from build123d import *

# Parameters (mm, degrees)
SKETCH1_W              = 200
SKETCH1_H              = 60
BOSS_EXTRUDE1_DEPTH    = 12
SKETCH2_W              = 16
SKETCH2_H              = 12
CUT_EXTRUDE1_DEPTH     = 106.090437243
SKETCH3_W              = 58
SKETCH3_H              = 28
CUT_EXTRUDE2_DEPTH     = 106.090437243
SKETCH4_W              = 58
SKETCH4_H              = 28
CUT_EXTRUDE3_DEPTH     = 106.090437243
SKETCH5_W              = 90
SKETCH5_H              = 5
M6_TAPPED_HOLE1_D      = 5
M6_TAPPED_HOLE1_DEPTH  = 13
M6_TAPPED_HOLE1_TIP    = 1.502151548
CHAMFER1_SIZE          = 1
CHAMFER2_SIZE          = 10
CHAMFER3_SIZE          = 5
FILLET1_R              = 10
M10_TAPPED_HOLE1_D     = 8.5
M10_TAPPED_HOLE1_DEPTH = 99.5
M10_TAPPED_HOLE1_TIP   = 2.553657631


with BuildPart() as part:
    # Sketch1 → Boss-Extrude1 (new body)
    with BuildSketch(Plane.XY.offset(6)):
        Rectangle(SKETCH1_W, SKETCH1_H)
    extrude(amount=-BOSS_EXTRUDE1_DEPTH)

    # Sketch2 → Cut-Extrude1 (cut, through all)
    with BuildSketch(Plane(origin=(0, 0, -6), x_dir=(-1, 0, 0), z_dir=(0, 0, -1))):
        with Locations((92, 0)):
            Rectangle(SKETCH2_W, SKETCH2_H)
    extrude(amount=-CUT_EXTRUDE1_DEPTH, mode=Mode.SUBTRACT)

    # Sketch3 → Cut-Extrude2 (cut, through all)
    with BuildSketch(Plane.XY.offset(6)):
        with Locations((-22, 0.2)):
            Rectangle(SKETCH3_W, SKETCH3_H)
    extrude(amount=-CUT_EXTRUDE2_DEPTH, mode=Mode.SUBTRACT)

    # Sketch4 → Cut-Extrude3 (cut, through all)
    with BuildSketch(Plane(origin=(0, 0, -6), x_dir=(-1, 0, 0), z_dir=(0, 0, -1))):
        with Locations((-58, 0.2)):
            Rectangle(SKETCH4_W, SKETCH4_H)
    extrude(amount=-CUT_EXTRUDE3_DEPTH, mode=Mode.SUBTRACT)

    # Sketch5 → Revolve1 (revolve)
    with BuildSketch(Plane(origin=(0, 0, 0), x_dir=(-1, 0, 0), z_dir=(0, 0, -1)), mode=Mode.PRIVATE) as revolve1_sk:
        with Locations((-145, 2.7)):
            Rectangle(SKETCH5_W, SKETCH5_H)
    revolve(revolve1_sk.sketch.rotate(Axis((190, 0.2, 0), (-1, 0, 0)), 270), axis=Axis((190, 0.2, 0), (-1, 0, 0)))

    # M6 Tapped Hole1
    with Locations(Plane.ZY.offset(100)):
        with Locations((0, 18)):
            Hole(M6_TAPPED_HOLE1_D / 2, depth=M6_TAPPED_HOLE1_DEPTH)
            with Locations((0, 0, -(M6_TAPPED_HOLE1_DEPTH + M6_TAPPED_HOLE1_TIP / 2))):  # 118° drill point
                Cone(0, M6_TAPPED_HOLE1_D / 2, M6_TAPPED_HOLE1_TIP, mode=Mode.SUBTRACT)

    # Chamfer1
    chamfer1_edges = [part.edges().sort_by_distance(p)[0] for p in [
        (190, 0.2, -5),
    ]]
    chamfer(chamfer1_edges, length=CHAMFER1_SIZE)

    # Chamfer2
    chamfer2_edges = [part.edges().sort_by_distance(p)[0] for p in [
        (100, 30, 0),
        (100, -30, 0),
    ]]
    chamfer(chamfer2_edges, length=CHAMFER2_SIZE)

    # Chamfer3
    chamfer3_edges = [part.edges().sort_by_distance(p)[0] for p in [
        (-100, -30, 0),
    ]]
    chamfer(chamfer3_edges, length=CHAMFER3_SIZE)

    # Fillet1
    fillet1_edges = [part.edges().sort_by_distance(p)[0] for p in [
        (-51, -13.8, 0),
        (-51, 14.2, 0),
        (7, 14.2, 0),
        (7, -13.8, 0),
        (29, 14.2, 0),
        (29, -13.8, 0),
        (87, -13.8, 0),
        (87, 14.2, 0),
    ]]
    fillet(fillet1_edges, radius=FILLET1_R)

    # M10 Tapped Hole1
    with Locations(Plane(origin=(190, 0, 0), x_dir=(0, 0, -1), z_dir=(1, 0, 0))):
        with Locations((0, 0.2)):
            Hole(M10_TAPPED_HOLE1_D / 2, depth=M10_TAPPED_HOLE1_DEPTH)
            with Locations((0, 0, -(M10_TAPPED_HOLE1_DEPTH + M10_TAPPED_HOLE1_TIP / 2))):  # 118° drill point
                Cone(0, M10_TAPPED_HOLE1_D / 2, M10_TAPPED_HOLE1_TIP, mode=Mode.SUBTRACT)


solid = part.part
The listing builds one solid part. Answer for the finished solid, in the listing's coordinates (mm). A direction names the side the tool comes from. Give positions to 0.01 mm unless a question says otherwise; leave off trailing zeros. Write each loop counter-clockwise with the first axis right and the second up, starting at its lowest first coordinate (ties: lowest second). Pieces come first, ordered by that corner, then holes.
Item 1: Which of the six approach directions +Z, -Z, +X, -X, +Y, -Y give full straight-line access (tool end or side, diameter ignored) to faces 1 (the flat face through (-84, 0, 0)), 2 (the flat face through (-22, -13.8, 0)), 3 (the flat face through (-6, 30, 0))?
Item 2: Determine the mould class of faces 4 (the flat face through (100, -5, 1)), 5 (the flat face through (95, -25, 0)), 6 (the cylindrical face through (-93.41, 20.48, 0.33)) for opening direction Y: released by +Y, released by -Y, zero draft, split by the parting line, or undercut.
Item 3: Section C-C, the plane y = -17.5 is taken. Write down the section's boundary in (x, z), plus the area to 3 significant figures.
Item 4: Section B-B, the plane x = 128 is taken. Write down the section's boundary in (y, z), plus the area to 3 significant figures.
Item 5: Find the intervals of material crossed by line 1 along X through (y, z) = (3.5, 5.25); line 2 along Y through (x, z) = (-23.5, -0.5); line 3 along X through (y, z) = (13, 2), in increasing order.
Item 6: Section A-A, the plane x = -27.5 is taken. Write down the section's boundary in (y, z).
Item 7: Flat-ended cylindrical pins translate along their axes: P1, Ø2, axis at x = 123, y = 3.5, coming from the -Z side; P2, Ø2.5, axis at y = 1, z = -1.5, coming from the -X side; P3, Ø1, axis at x = 115.5, y = 7, coming from the +Z side; P4, Ø6, axis at y = 18, z = 0, coming from the +X side. Find the tip coordinate at first contact, or state that the pin passes through.
Completed:
1. face 1: +Z, -Z, -X
1. face 2: +Z, -Z
1. face 3: +Z, -Z, +X, -X, +Y
2. face 4: zero draft
2. face 5: released by -Y
2. face 6: undercut
3. outline: (-100, -6) - (100, -6) - (100, 6) - (-100, 6) - close
3. area: 2,400 mm2
4. outline: circle Ø10 at (0.2, 0); hole circle Ø8.5 at (0.2, 0)
4. area: 21.8 mm2
5. line 1: x = -84 to -51, 7 to 29, 87 to 100
5. line 2: y = -30 to -13.8, 14.2 to 30
5. line 3: x = -100 to -45.75, 1.75 to 34.25, 81.75 to 100
6. outline: (-30, -6) - (-13.8, -6) - (-13.8, 6) - (-30, 6) - close; (14.2, -6) - (30, -6) - (30, 6) - (14.2, 6) - close
7. P1: stops at z = -4.44
7. P2: stops at x = -84
7. P3: passes through
7. P4: stops at x = 100
